```python
from build123d import *

# Parameters (mm, degrees)
SKETCH1_R           = 12.5
BOSS_EXTRUDE1_DEPTH = 10
SKETCH2_R           = 14
BOSS_EXTRUDE2_DEPTH = 300


with BuildPart() as part:
    # Sketch1 → Boss-Extrude1 (new body)
    with BuildSketch(Plane(origin=(0, 0, 0), x_dir=(1, 0, 0), z_dir=(0, 1, 0))):
        with BuildLine():
            Line((36.142857143, 20), (72.285714286, 20))
            ThreePointArc((72.285714286, 20), (92.285714286, 0), (72.285714286, -20))
            Line((72.285714286, -20), (36.142857143, -20))
            Line((36.142857143, -20), (36.142857143, 20))
        make_face()
        with Locations(Location((72.285714286, 0, 0), (0, 0, 270))):
            Circle(SKETCH1_R, mode=Mode.SUBTRACT)
    boss_extrude1 = extrude(amount=BOSS_EXTRUDE1_DEPTH)

    # Sketch2 → Boss-Extrude2 (add)
    with BuildSketch(Plane.ZY.offset(-36.142857143)):
        with Locations(Location((0, -10, 0), (0, 0, 134.415308597))):
            Circle(SKETCH2_R)
    extrude(amount=BOSS_EXTRUDE2_DEPTH)

    # Mirror1: Boss-Extrude1 across plane
    add(boss_extrude1.mirror(Plane(origin=(0, -10, 0), x_dir=(0, 0, 1), z_dir=(0, -1, 0))))


solid = part.part
```
Could you check a few things on this model? Use its own coordinates, in mm. A direction names the side the tool comes from. Give positions to 0.01 mm unless a question says otherwise; leave off trailing zeros. Loops run counter-clockwise (first coordinate to the right, second up) from the corner with the lowest first, then second, coordinate; pieces in that order, holes last. Notation, with made-up numbers: (-22.75, 81) - (-15.75, 81) arc R24 ccw to (-15.75, 99) - close; hole circle Ø8 at (69, 0.25). An arc over 180 degrees is marked (long way). Answer in a Markdown table with one row per item. Add a question column.
Q1. Which directions (+Z, -Z, +X, -X, +Y, -Y) give clear straight access to the entire face, cutting with the end or side of a thin tool? Please do faces 4 (the face through (-112, -24, 0)), 5 (the face through (58, -30, 0)), 6 (the face through (36.143, -26, 0)), 7 (the face through (58, -20, 0)), 8 (the face through (36.143, 6, 0)).
Q2. For pin 1 (6 mm diameter, centred on x = -224.5, z = -6.5, fed in from +Y); pin 2 (3 mm diameter, centred on y = -25.5, z = -3.5, fed in from -X); pin 3 (8 mm diameter, centred on y = -8.5, z = -10, fed in from +X), each with a flat end and sliding along its axis, tell me the tip position at first contact or that it passes through.
Q3. If we section it at A-A (z = 0): List the corners of the cut face in (x, y) for me, plus the area to 3 significant figures.
Q4. Please list where these lines run through material, in increasing order: L1, parallel to X at y = -27, z = -0.5; L2, parallel to X at y = -7, z = 9.5; L3, parallel to X at y = -22.75, z = 0. Write a range as from..to.
Q5. We'd pull the mould along X, two halves only. Please class faces 1 (the face through (92.28, 4.93, -0.44)), 2 (the face through (60.083, -24.93, -2.71)), 3 (the face through (54, 5, -20)): +X half, -X half, draft (parallel to the pull), parting line (faces both ways), or undercut.
Q6. If we section it at C-C (x = -104): List the corners of the cut face in (y, z) for me.
Q7. If we section it at B-B (y = -10): List the corners of the cut face in (x, z) for me, plus the area to 3 significant figures.
The answers:
| question | item | result |
|---|---|---|
| 1 | face 4 | -X |
| 1 | face 5 | +Z, -Z, +X, -X, -Y |
| 1 | face 6 | -X, -Y |
| 1 | face 7 | +Z, -Z, +X |
| 1 | face 8 | -X, +Y |
| 2 | pin 1 | stops at y = 3.56 |
| 2 | pin 2 | stops at x = 36.14 |
| 2 | pin 3 | stops at x = 36.14 |
| 3 | outline | (-263.86, -24) - (36.14, -24) - (36.14, -30) - (59.79, -30) - (59.79, -20) - (36.14, -20) - (36.14, 0) - (59.79, 0) - (59.79, 10) - (36.14, 10) - (36.14, 4) - (-263.86, 4) - close; (84.79, -30) - (92.29, -30) - (92.29, -20) - (84.79, -20) - close; (84.79, 0) - (92.29, 0) - (92.29, 10) - (84.79, 10) - close |
| 3 | area | 9,020 mm^2 |
| 4 | L1 | x = 36.14..59.8, 84.78..92.28 |
| 4 | L2 | x = -263.86..36.14 |
| 4 | L3 | x = -263.86..59.79, 84.79..92.29 |
| 5 | face 1 | +X half |
| 5 | face 2 | undercut |
| 5 | face 3 | draft |
| 6 | outline | circle Ø28 at (-10, 0) |
| 7 | outline | (-263.86, -14) - (36.14, -14) - (36.14, 14) - (-263.86, 14) - close |
| 7 | area | 8,400 mm^2 |
